Verification items for this drawing (mm, ordinates from the low corner). A direction names the side the tool comes from. Round coordinates to 2 decimals unless told otherwise and drop trailing zeros. Order: outer loops, then holes, each group sorted by start corner. A loop starts at its lowest first (then second) coordinate and runs counter-clockwise, first axis right, second up. Notation, with made-up numbers: (84.5, 63.25) - (110.5, 63.25) arc R18 ccw to (110.5, 71.25) - close; hole circle Ø8 at (16, 52.25). An arc over 180 degrees is marked (long way). Use a Markdown table: item, result. Add a question column.
(1) Thickness scan on line 1 along Z through (x, y) = (0.65, 2.95); line 2 along Z through (x, y) = (2.5, 0.3); line 3 along X through (y, z) = (3.5, 2). Record the ranges inside material, lowest first. Write a range as [from, to].
(2) Section check C-C on z = 2. Record the boundary of the cut face in (x, y).
(3) Gauge pin test, flat ends, axial feed: P1, Ø1.5, axis at y = 2, z = 7, coming from the -X side; P2, Ø1.2, axis at y = 2, z = 1.5, coming from the +X side; P3, Ø3, axis at y = 3.5, z = 3, coming from the -X side. Record the tip position at first contact, or that the pin passes through.
(4) Section check A-A on x = 2.5. Record the boundary of the cut face in (y, z), then the cut area to 3 significant figures.
(5) Mould release check, pull along Z, two halves, no side actions. Record for the marked faces 1, 2, 3 and 4: released by +Z, released by -Z, zero draft, split by the parting line, or undercut.
(6) Section check D-D on y = 3.2. Record the boundary of the cut face in (x, z).
(7) Access from +Z, -Z, +X, -X, +Y, -Y to the whole of each face (thin tool, end or side, straight path). Record for the marked faces 5, 6, 7 and 8.
(8) Section check B-B on y = 2.5. Record the boundary of the cut face in (x, z), then the cut area to 3 significant figures.
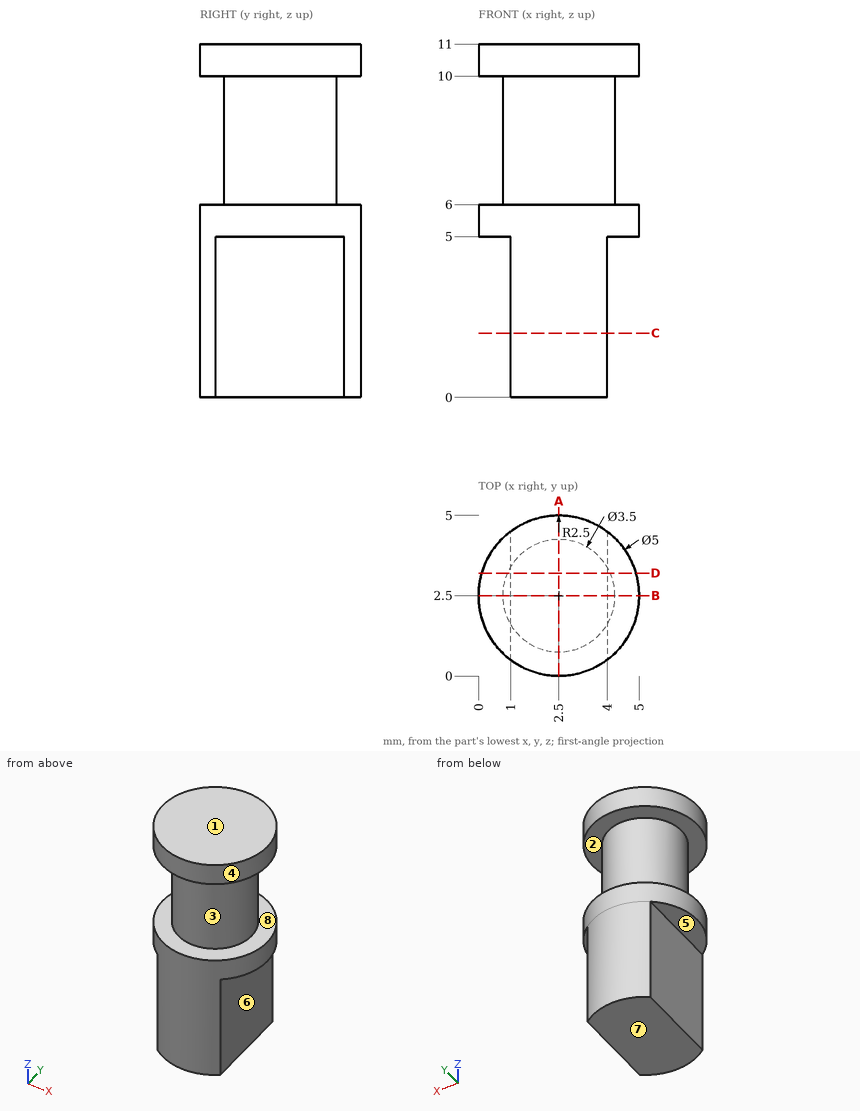
Check sheet entries:
| question | item | result |
|---|---|---|
| 1 | line 1 | z = [5, 6], [10, 11] |
| 1 | line 2 | z = [0, 6], [10, 11] |
| 1 | line 3 | x = [1, 4] |
| 2 | outline | (1, 0.5) arc R2.5 ccw to (4, 0.5) - (4, 4.5) arc R2.5 ccw to (1, 4.5) - close |
| 3 | P1 | stops at x = 0.75 |
| 3 | P2 | stops at x = 4 |
| 3 | P3 | stops at x = 1 |
| 4 | outline | (0, 0) - (5, 0) - (5, 6) - (4.25, 6) - (4.25, 10) - (5, 10) - (5, 11) - (0, 11) - (0, 10) - (0.75, 10) - (0.75, 6) - (0, 6) - close |
| 4 | area | 49.0 mm2 |
| 5 | face 1 | released by +Z |
| 5 | face 2 | undercut |
| 5 | face 3 | undercut |
| 5 | face 4 | zero draft |
| 6 | outline | (0.1, 5) - (1, 5) - (1, 0) - (4, 0) - (4, 5) - (4.9, 5) - (4.9, 6) - (4.1, 6) - (4.1, 10) - (4.9, 10) - (4.9, 11) - (0.1, 11) - (0.1, 10) - (0.9, 10) - (0.9, 6) - (0.1, 6) - close |
| 7 | face 5 | -Z, -X, +Y, -Y |
| 7 | face 6 | -Z, +X, +Y, -Y |
| 7 | face 7 | -Z, +X, -X, +Y, -Y |
| 7 | face 8 | none |
| 8 | outline | (0, 5) - (1, 5) - (1, 0) - (4, 0) - (4, 5) - (5, 5) - (5, 6) - (4.25, 6) - (4.25, 10) - (5, 10) - (5, 11) - (0, 11) - (0, 10) - (0.75, 10) - (0.75, 6) - (0, 6) - close |
| 8 | area | 39.0 mm2 |
